Input: part model. Units: mm. Frame: model coordinates. Face numbers are marked on the shaded views. Round coordinates to 2 decimals unless told otherwise and drop trailing zeros. Write each loop counter-clockwise with the first axis right and the second up, starting at its lowest first coordinate (ties: lowest second). Pieces come first, ordered by that corner, then holes. Notation, with made-up numbers: (-34.75, 72.25) -> (-21.75, 72.25) arc R12 cw to (-21.75, 87.25) -> close; hole circle Ø11 at (18, -38). An arc over 180 degrees is marked (long way). Write item = value, one per line.
```python
from build123d import *

# Parameters (mm, degrees)
SKETCH1_W                  = 24
SKETCH1_H                  = 4
BOSS_EXTRUDE1_DEPTH        = 0.75
F_2_3_2_3_DIAMETER_HOLE1_D = 2.3


with BuildPart() as part:
    # Sketch1 → Boss-Extrude1 (new, symmetric)
    with BuildSketch(Plane(origin=(0, 0, 0), x_dir=(1, 0, 0), z_dir=(0, 1, 0))):
        Rectangle(SKETCH1_W, SKETCH1_H)
    extrude(amount=BOSS_EXTRUDE1_DEPTH, both=True)

    # Ø2.3 (2.3) Diameter Hole1 (through all)
    with Locations(Plane(origin=(0, 0.75, 0), x_dir=(1, 0, 0), z_dir=(0, 1, 0))):
        with Locations((-9.5, 0), (9.5, 0)):
            Hole(F_2_3_2_3_DIAMETER_HOLE1_D / 2)


solid = part.part
```
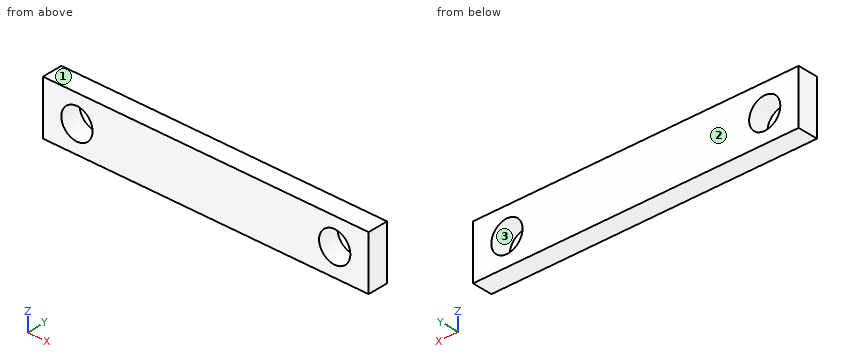
1) Line query: L1, parallel to X at y = 0.7, z = -0.05; L2, parallel to X at y = -0.1, z = -0.7; L3, parallel to Z at x = 9.5, y = 0.4. Output: solid intervals per line, ascending. Write a range as from..to.
Solutions:
L1 = -12..-10.65, -8.35..8.35, 10.65..12
L2 = -12..-10.41, -8.59..8.59, 10.41..12
L3 = -2..-1.15, 1.15..2
2) Cut plane C-C (x = -9.5). Return the cut outline in (y, z), and give its area (3 significant figures).
Solutions:
outline = (-0.75, -2) -> (0.75, -2) -> (0.75, -1.15) -> (-0.75, -1.15) -> close; (-0.75, 1.15) -> (0.75, 1.15) -> (0.75, 2) -> (-0.75, 2) -> close
area = 2.55 mm^2
3) Cut plane A-A (z = 0). Return the cut outline in (x, y).
Solutions:
outline = (-12, -0.75) -> (-10.65, -0.75) -> (-10.65, 0.75) -> (-12, 0.75) -> close; (-8.35, -0.75) -> (8.35, -0.75) -> (8.35, 0.75) -> (-8.35, 0.75) -> close; (10.65, -0.75) -> (12, -0.75) -> (12, 0.75) -> (10.65, 0.75) -> close
4) Draft query along Z for the marked faces 1, 2 and 3. Return one class per face: +Z half, -Z half, draft (parallel to the pull), parting line (faces both ways), or undercut.
Solutions:
face_1 = +Z half
face_2 = draft
face_3 = undercut
5) Cut plane D-D (z = -0.95). Return the cut outline in (x, y), and give its area (3 significant figures).
Solutions:
outline = (-12, -0.75) -> (-10.15, -0.75) -> (-10.15, 0.75) -> (-12, 0.75) -> close; (-8.85, -0.75) -> (8.85, -0.75) -> (8.85, 0.75) -> (-8.85, 0.75) -> close; (10.15, -0.75) -> (12, -0.75) -> (12, 0.75) -> (10.15, 0.75) -> close
area = 32.1 mm^2
6) Cut plane B-B (y = -0.05). Return the cut outline in (x, z).
Solutions:
outline = (-12, -2) -> (12, -2) -> (12, 2) -> (-12, 2) -> close; hole circle Ø2.3 at (-9.5, 0); hole circle Ø2.3 at (9.5, 0)
